from build123d import *

# Parameters (mm, degrees)
SKETCH1_R          = 40
EXTRUDE1_DEPTH     = 20
SKETCH2_R          = 12
CUT_EXTRUDE1_DEPTH = 61
CHAMFER1_SIZE      = 1
CHAMFER2_SIZE      = 5.5
CHAMFER2_SIZE2     = 3.175426481


with BuildPart() as part:
    # Sketch1 → Extrude1 (new body)
    with BuildSketch(Plane(origin=(0, 0, 0), x_dir=(0, 0, -1), z_dir=(1, 0, 0))):
        Circle(SKETCH1_R)
    extrude(amount=EXTRUDE1_DEPTH)

    # Sketch2 → Cut-Extrude1 (cut, through all)
    with BuildSketch(Plane(origin=(20, 0, 0), x_dir=(0, 0, -1), z_dir=(1, 0, 0))):
        Circle(SKETCH2_R)
    extrude(amount=-CUT_EXTRUDE1_DEPTH, mode=Mode.SUBTRACT)

    # Chamfer1
    chamfer1_edges = [part.edges().sort_by_distance(p)[0] for p in [
        (0, 0, 40),
        (20, 0, 40),
    ]]
    chamfer(chamfer1_edges, length=CHAMFER1_SIZE)

    # Chamfer2
    chamfer2_edges = [part.edges().sort_by_distance(p)[0] for p in [
        (20, 0, 12),
    ]]
    chamfer2_side = [part.faces().sort_by_distance(p)[0] for p in [
        (20, 0, 37.896913421),
    ]]
    chamfer(chamfer2_edges, length=CHAMFER2_SIZE, length2=CHAMFER2_SIZE2, reference=chamfer2_side[0])


solid = part.part
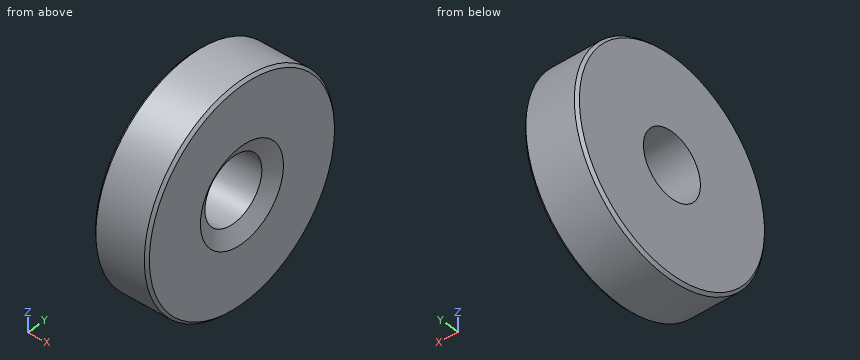
Work out the finished part from the listing and answer in its coordinate system (mm). Give positions to 0.01 mm unless a question says otherwise; leave off trailing zeros. Order: outer loops, then holes, each group sorted by start corner. A loop starts at its lowest first (then second) coordinate and runs counter-clockwise, first axis right, second up. Notation, with made-up numbers: M -13,57.5 L 29,57.5 A23 ccw 29,82.5 Z; hole C 78.25,52.25 d6. An arc over 180 degrees is marked long. Return JSON: item names as keys, results as strings.
Q1. Each of these flat-tipped pins is pushed along its axis until it touches: pin 1 (10 mm diameter, centred on x = 10.5, z = -8.5, fed in from -Y); pin 2 (5 mm diameter, centred on x = 14, z = 23.5, fed in from +Y); pin 3 (3 mm diameter, centred on x = 7.5, y = 29.5, fed in from -Z); pin 4 (21.5 mm diameter, centred on y = 0, z = 0, fed in from +X). Where does it stop, or does it pass through?
Answer below:
{"pin 1": "stops at y = -39.85", "pin 2": "stops at y = 34.04", "pin 3": "stops at z = -28.57", "pin 4": "passes through"}
Q2. Find section A-A, the plane y = 0. Write down the section's boundary in (x, z), and give its area (3 significant figures).
Answer below:
{"outline": "M 0,-39 L 1,-40 L 19,-40 L 20,-39 L 20,-17.5 L 16.82,-12 L 0,-12 Z; M 0,12 L 16.82,12 L 20,17.5 L 20,39 L 19,40 L 1,40 L 0,39 Z", "area": "1,100 mm^2"}
Q3. Find section C-C, the plane x = 9.5. Write down the section's boundary in (y, z), and give its area (3 significant figures).
Answer below:
{"outline": "C 0,0 d80; hole C 0,0 d24", "area": "4,570 mm^2"}
Q4. Find the intervals of material crossed by line 1 along Y through (x, z) = (5.25, 0); line 2 along Y through (x, z) = (1.5, 1.5); line 3 along Z through (x, y) = (14.5, 2.5), in increasing order. Write a range as [from, to].
Answer below:
{"line 1": "y = [-40, -12], [12, 40]", "line 2": "y = [-39.97, -11.91], [11.91, 39.97]", "line 3": "z = [-39.92, -11.74], [11.74, 39.92]"}
